Geometry: final body of the model. Coordinates: model frame, mm. Face numbers are marked on the shaded views. Round coordinates to 2 decimals unless told otherwise and drop trailing zeros. Order: outer loops, then holes, each group sorted by start corner. A loop starts at its lowest first (then second) coordinate and runs counter-clockwise, first axis right, second up. Notation, with made-up numbers: M 77.25,61 L 115.25,61 A14 ccw 115.25,79 Z; hole C 40.25,89.5 d6. An arc over 180 degrees is marked long. Put each result on its own line as item: value. Start each with the question number.
1) Section B-B, the plane z = 4.25. Return loops of the section in (x, y).
2) First-contact query: P1, Ø11, axis at x = -10, y = 0, coming from the -Z side. Flat tip, straight axial feed; report the tip coordinate or a pass-through.
3) Material intervals for probe 1 along Y at (x, z) = (-10, 0.25); probe 2 along X at (y, z) = (-2, 2.25); probe 3 along Y at (x, z) = (-9, -3.5), sorted ascending. Write a range as [from, to].
4) Section A-A, the plane x = -10. Return loops of the section in (y, z).
5) Draft query along X for the marked faces 1, 2 and 3. Return one class per face: pulls with the +X half, pulls with the -X half, needs draft (parallel to the pull), parting line crosses it, or undercut.
6) Section C-C, the plane y = 0. Return loops of the section in (x, z), then the cut area to 3 significant figures.
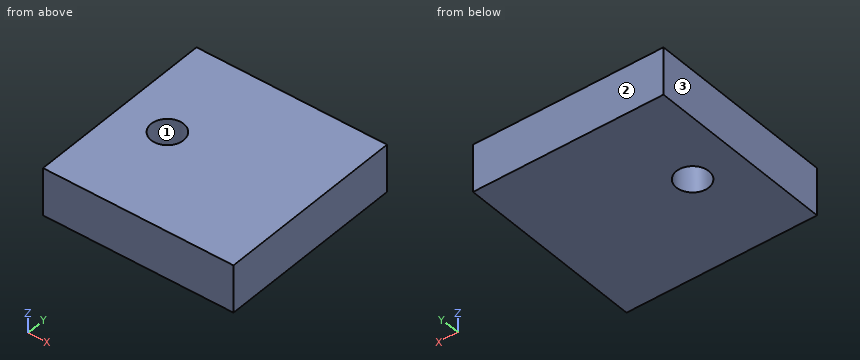
from build123d import *

# Parameters (mm, degrees)
SKETCH_1_W         = 40
SKETCH_1_H         = 40
EXTRUDE_1_DEPTH    = 5
HOLE_WIZARD_M8_1_D = 6.8


with BuildPart() as part:
    # 草图1 → 凸台-拉伸1 (new, symmetric)
    with BuildSketch(Plane.XY):
        Rectangle(SKETCH_1_W, SKETCH_1_H)
    extrude(amount=EXTRUDE_1_DEPTH, both=True)

    # M8 螺纹孔1 (through all)
    with Locations(Plane.XY.offset(5)):
        with Locations((-10, 0)):
            Hole(HOLE_WIZARD_M8_1_D / 2)


solid = part.part
Result sheet:
1. outline: M -20,-20 L 20,-20 L 20,20 L -20,20 Z; hole C -10,0 d6.8
2. P1: stops at z = -5
3. probe 1: y = [-20, -3.4], [3.4, 20]
3. probe 2: x = [-20, -12.75], [-7.25, 20]
3. probe 3: y = [-20, -3.25], [3.25, 20]
4. outline: M -20,-5 L -3.4,-5 L -3.4,5 L -20,5 Z; M 3.4,-5 L 20,-5 L 20,5 L 3.4,5 Z
5. face 1: undercut
5. face 2: needs draft
5. face 3: pulls with the -X half
6. outline: M -20,-5 L -13.4,-5 L -13.4,5 L -20,5 Z; M -6.6,-5 L 20,-5 L 20,5 L -6.6,5 Z
6. area: 332 mm2
